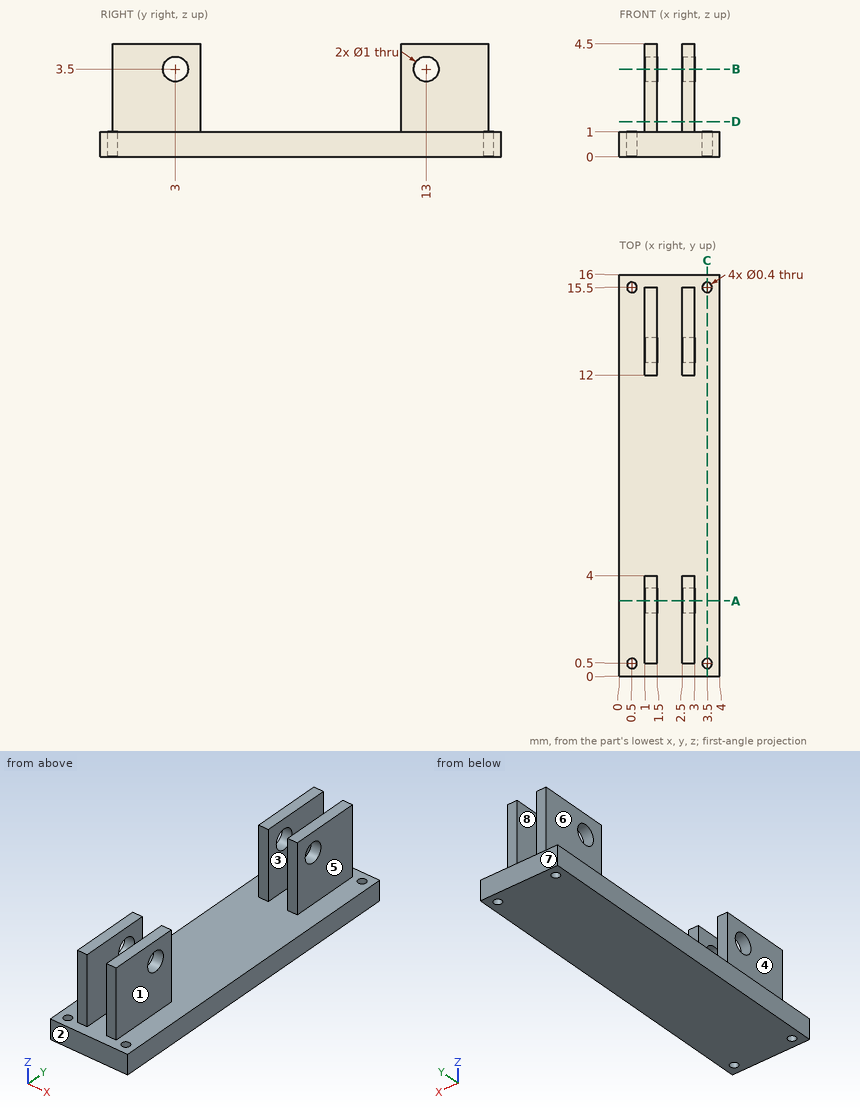
Job drawing, mm, ordinate dimensions from the low corner. One solid piece. A direction names the side the tool comes from. Give positions to 0.01 mm unless a question says otherwise; leave off trailing zeros. Order: outer loops, then holes, each group sorted by start corner. A loop starts at its lowest first (then second) coordinate and runs counter-clockwise, first axis right, second up. Notation, with made-up numbers: (-27, -3.5) - (-21, -3.5) arc R17 ccw to (-21, 25.5) - close; hole circle Ø3 at (32, 67.5). An arc over 180 degrees is marked (long way). Answer in a Markdown table with one row per item.
1. Saw through at A-A, the plane y = 3. Give the cut face in (x, z), plus the area to 3 significant figures.
Data:
| item | result |
|---|---|
| outline | (0, 0) - (4, 0) - (4, 1) - (3, 1) - (3, 3) - (2.5, 3) - (2.5, 1) - (1.5, 1) - (1.5, 3) - (1, 3) - (1, 1) - (0, 1) - close; (1, 4) - (1.5, 4) - (1.5, 4.5) - (1, 4.5) - close; (2.5, 4) - (3, 4) - (3, 4.5) - (2.5, 4.5) - close |
| area | 6.50 mm² |
2. Tool access for the marked faces 1, 2, 3 and 4: list every direction of +Z, -Z, +X, -X, +Y, -Y with a clear straight run to the whole face (end or side of a thin tool).
Data:
| item | result |
|---|---|
| face 1 | +Z, +X, +Y, -Y |
| face 2 | +Z, -Z, +X, -X, -Y |
| face 3 | +Z, +Y, -Y |
| face 4 | +Z, -X, +Y, -Y |
3. Saw through at C-C, the plane x = 3.5. Give the cut face in (y, z).
Data:
| item | result |
|---|---|
| outline | (0, 0) - (0.3, 0) - (0.3, 1) - (0, 1) - close; (0.7, 0) - (15.3, 0) - (15.3, 1) - (0.7, 1) - close; (15.7, 0) - (16, 0) - (16, 1) - (15.7, 1) - close |
4. Flat gauge pins, fed straight in: pin 1 (1.5 mm diameter, centred on x = 3, z = 2.5, fed in from +Y); pin 2 (1 mm diameter, centred on y = 2.5, z = 2, fed in from +X); pin 3 (0.6 mm diameter, centred on x = 1, z = 3.5, fed in from -Y). Where does each tip first touch, or does it go through?
Data:
| item | result |
|---|---|
| pin 1 | stops at y = 15.5 |
| pin 2 | stops at x = 3 |
| pin 3 | stops at y = 0.5 |
5. Probe probe 1 along Y at (x, z) = (1.3, 3.5); probe 2 along Y at (x, z) = (3.5, 0.8); probe 3 along X at (y, z) = (0.5, 0.7). List the from-to ranges inside material, lowest first. Write a range as [from, to].
Data:
| item | result |
|---|---|
| probe 1 | y = [0.5, 2.5], [3.5, 4], [12, 12.5], [13.5, 15.5] |
| probe 2 | y = [0, 0.3], [0.7, 15.3], [15.7, 16] |
| probe 3 | x = [0, 0.3], [0.7, 3.3], [3.7, 4] |
6. Pull direction X, two halves, no side cores. Call the marked faces 5, 6, 7 and 8: pulls with the +X half, pulls with the -X half, needs draft (parallel to the pull), parting line crosses it, or undercut.
Data:
| item | result |
|---|---|
| face 5 | pulls with the +X half |
| face 6 | pulls with the -X half |
| face 7 | needs draft |
| face 8 | undercut |
7. Saw through at D-D, the plane z = 1.4. Give the cut face in (x, y).
Data:
| item | result |
|---|---|
| outline | (1, 0.5) - (1.5, 0.5) - (1.5, 4) - (1, 4) - close; (1, 12) - (1.5, 12) - (1.5, 15.5) - (1, 15.5) - close; (2.5, 0.5) - (3, 0.5) - (3, 4) - (2.5, 4) - close; (2.5, 12) - (3, 12) - (3, 15.5) - (2.5, 15.5) - close |
8. Saw through at B-B, the plane z = 3.5. Count the separate pieces of the cut face and the enclosed holes in it, plus the area to 3 significant figures.
Data:
| item | result |
|---|---|
| separate pieces | 8 |
| enclosed holes | 0 |
| area | 5.00 mm² |
